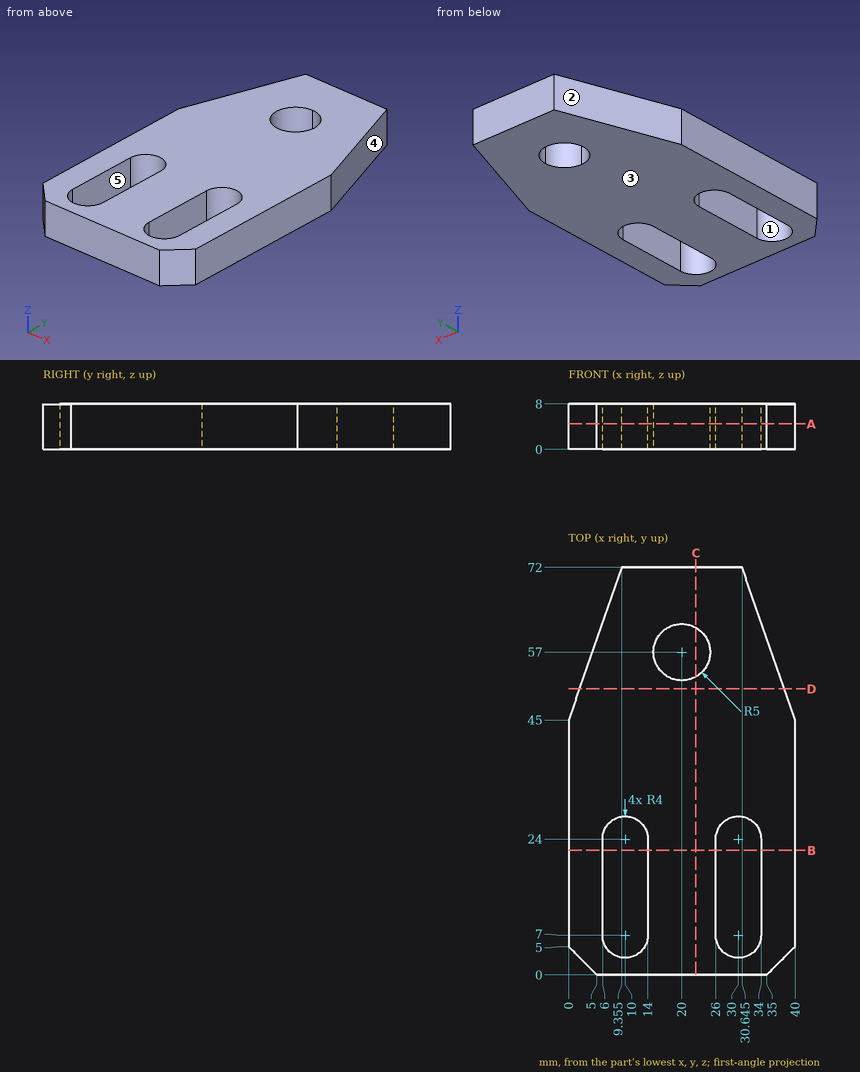
Print and shaded views of the part. All mm, measured from the part's lowest x, y and z. A direction names the side the tool comes from. Round coordinates to 2 decimals unless told otherwise and drop trailing zeros. Write each loop counter-clockwise with the first axis right and the second up, starting at its lowest first coordinate (ties: lowest second). Pieces come first, ordered by that corner, then holes. Notation, with made-up numbers: (17.5, 84) - (23.5, 84) arc R20 ccw to (23.5, 92) - close; hole circle Ø6 at (-4, 26.25). An arc over 180 degrees is marked (long way). Write each question's results on one line, items separated by ' | '. Start each with the question number.
Item 1: Wall check: L1, parallel to X at y = 16.5, z = 0.75; L2, parallel to X at y = 5.5, z = 1.5; L3, parallel to Y at x = 24, z = 6. Give the ranges that are in metal, low to high. Write a range as [from, to].
Item 2: Saw through at B-B (y = 22). Write the cut outline in (x, z), and give its area (3 significant figures).
Item 3: Saw through at C-C (x = 22.5). Write the cut outline in (y, z), and give its area (3 significant figures).
Item 4: Saw through at D-D (y = 50.5). Write the cut outline in (x, z).
Item 5: Mould opens along X. For the marked faces 3, 4 and 5 say: pulls with the +X half, pulls with the -X half, needs draft (parallel to the pull), parting line crosses it, or undercut.
Item 6: Saw through at A-A (z = 4.5). Write the cut outline in (x, y) (3 decimals).
Item 7: Which spindle directions (+Z, -Z, +X, -X, +Y, -Y) get a long thin tool onto all of the face, cutting with end or side? Do the marked faces 1 and 2. Say none if no direction does.
Results are:
1) L1: x = [0, 6], [14, 26], [34, 40] | L2: x = [0, 6.29], [13.71, 26.29], [33.71, 40] | L3: y = [0, 54], [60, 72]
2) outline: (0, 0) - (6, 0) - (6, 8) - (0, 8) - close; (14, 0) - (26, 0) - (26, 8) - (14, 8) - close; (34, 0) - (40, 0) - (40, 8) - (34, 8) - close | area: 192 mm²
3) outline: (0, 0) - (52.67, 0) - (52.67, 8) - (0, 8) - close; (61.33, 0) - (72, 0) - (72, 8) - (61.33, 8) - close | area: 507 mm²
4) outline: (1.91, 0) - (38.09, 0) - (38.09, 8) - (1.91, 8) - close
5) face 3: needs draft | face 4: pulls with the +X half | face 5: undercut
6) outline: (0, 5) - (5, 0) - (35, 0) - (40, 5) - (40, 45) - (30.645, 72) - (9.355, 72) - (0, 45) - close; hole (6, 7) arc R4 ccw to (14, 7) - (14, 24) arc R4 ccw to (6, 24) - close; hole circle Ø10 at (20, 57); hole (26, 7) arc R4 ccw to (34, 7) - (34, 24) arc R4 ccw to (26, 24) - close
7) face 1: +Z, -Z | face 2: +Z, -Z, -X, +Y
